from build123d import *

# Parameters (mm, degrees)
SKETCH1_R           = 30
BOSS_EXTRUDE1_DEPTH = 25
SKETCH2_R           = 43.5
BOSS_EXTRUDE2_DEPTH = 100


with BuildPart() as part:
    # Sketch1 → Boss-Extrude1 (new, symmetric)
    with BuildSketch(Plane(origin=(0, 0, 0), x_dir=(0, 0, -1), z_dir=(1, 0, 0))):
        with BuildLine():
            Line((-65.5, 170), (-59, 0))
            Line((-59, 0), (59, 0))
            Line((59, 0), (65.5, 170))
            ThreePointArc((65.5, 170), (0, 235.5), (-65.5, 170))
        make_face()
        with Locations((0, 170)):
            Circle(SKETCH1_R, mode=Mode.SUBTRACT)
    extrude(amount=BOSS_EXTRUDE1_DEPTH, both=True)

    # Sketch2 → Boss-Extrude2 (add)
    with BuildSketch(Plane(origin=(0, 0, 0), x_dir=(1, 0, 0), z_dir=(0, 1, 0))):
        Circle(SKETCH2_R)
    extrude(amount=BOSS_EXTRUDE2_DEPTH)


solid = part.part
Input: part model. Units: mm. Frame: model coordinates. A direction names the side the tool comes from. Give positions to 0.01 mm unless a question says otherwise; leave off trailing zeros. Write each loop counter-clockwise with the first axis right and the second up, starting at its lowest first coordinate (ties: lowest second). Pieces come first, ordered by that corner, then holes.
Q1. Set-up query: faces 4 (the face through (-32, 100, 0)), 5 (the face through (43.496, 49.3, 0.584)), 6 (the face through (32, 100, 0)), 7 (the face through (25, 119, 1)), 8 (the face through (-25, 119, 1)). Return all of +Z, -Z, +X, -X, +Y, -Y with unobstructed straight access to the full face (end or side cutting, diameter ignored); none if empty.
Q2. Section A-A, the plane z = 0. Output: boundary loops of the cut face in (x, y).
Q3. Section D-D, the plane y = 85. Output: boundary loops of the cut face in (x, z), plus the area to 3 significant figures.
Q4. Section B-B, the plane y = 159. Output: boundary loops of the cut face in (x, z).
Q5. Section C-C, the plane x = -21.5. Output: boundary loops of the cut face in (y, z), plus the area to 3 significant figures.
Q6. First-contact query: P1, Ø9.5, axis at x = 29.5, z = 6, coming from the +Y side; P2, Ø1.5, axis at x = 7.5, y = 29.5, coming from the +Z side; P3, Ø5.5, axis at x = -39, z = 7, coming from the +Y side. Flat tips, straight axial feed; report the tip coordinate or a pass-through.
Q7. Material intervals for probe 1 along Y at (x, z) = (-9, 0); probe 2 along X at (y, z) = (148, 57.5); probe 3 along Z at (x, y) = (-15, 177), sorted ascending.
Q8. Pull-direction query (Y, two-part tool) for faces 1 (the face through (-1, 0, -1)), 2 (the face through (-0.35, 140.713, 6.503)), 3 (the face through (0.35, 235.484, -1.44)); classes: pulls with the +Y half, pulls with the -Y half, needs draft (parallel to the pull), parting line crosses it, or undercut.
Filled in:
1. face 4: +Z, -Z, -X, +Y
1. face 5: +X, +Y, -Y
1. face 6: +Z, -Z, +X, +Y
1. face 7: +X, +Y
1. face 8: -X, +Y
2. outline: (-43.5, 0) - (43.5, 0) - (43.5, 100) - (25, 100) - (25, 140) - (-25, 140) - (-25, 100) - (-43.5, 100) - close; (-25, 200) - (25, 200) - (25, 235.5) - (-25, 235.5) - close
3. outline: (-25, -62.25) - (25, -62.25) - (25, -35.6) arc R43.5 ccw to (25, 35.6) - (25, 62.25) - (-25, 62.25) - (-25, 35.6) arc R43.5 ccw to (-25, -35.6) - close
3. area: 8,070 mm2
4. outline: (-25, -65.08) - (25, -65.08) - (25, -27.91) - (-25, -27.91) - close; (-25, 27.91) - (25, 27.91) - (25, 65.08) - (-25, 65.08) - close
5. outline: (0, -59) - (170, -65.5) arc R65.5 ccw to (170, 65.5) - (0, 59) - close; hole circle Ø60 at (170, 0)
5. area: 25,100 mm2
6. P1: stops at y = 235.35
6. P2: stops at z = 60.16
6. P3: stops at y = 100
7. probe 1: y = 0 to 140, 200 to 235.5
7. probe 2: x = -25 to 25
7. probe 3: z = -65.12 to -29.17, 29.17 to 65.12
8. face 1: pulls with the -Y half
8. face 2: undercut
8. face 3: pulls with the +Y half
